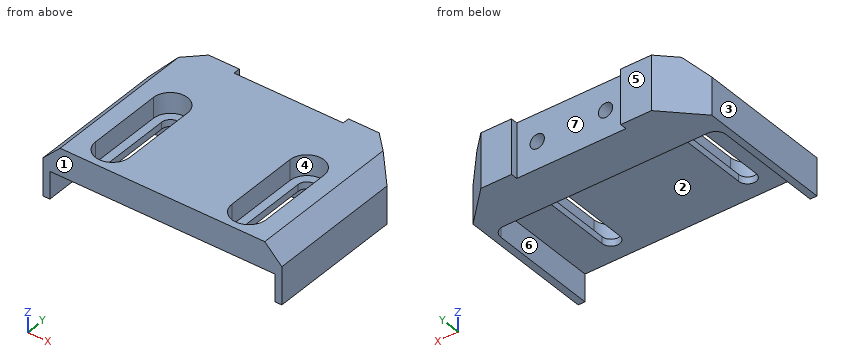
```python
from build123d import *

# Parameters (mm, degrees)
SKETCH1_W             = 70
SKETCH1_H             = 50
EXTRUDE1_DEPTH        = 8
SKETCH2_W             = 32
SKETCH2_H             = 16
EXTRUDE2_DEPTH        = 2
M5_TAPPED_HOLE1_D     = 4.2
M5_TAPPED_HOLE1_DEPTH = 8.4
M5_TAPPED_HOLE1_TIP   = 1.2618073
EXTRUDE3_DEPTH        = 8
EXTRUDE4_DEPTH        = 46.891175622
EXTRUDE5_DEPTH        = 6
CHAMFER1_SIZE         = 10
CHAMFER2_SIZE         = 5


with BuildPart() as part:
    # Sketch1 → Extrude1 (new, symmetric)
    with BuildSketch(Plane.XY):
        Rectangle(SKETCH1_W, SKETCH1_H)
    extrude(amount=EXTRUDE1_DEPTH, both=True)

    # Sketch2 → Extrude2 (cut)
    with BuildSketch(Plane(origin=(0, 25, 0), x_dir=(1, 0, 0), z_dir=(0, 1, 0))):
        Rectangle(SKETCH2_W, SKETCH2_H)
    extrude(amount=-EXTRUDE2_DEPTH, mode=Mode.SUBTRACT)

    # M5 Tapped Hole1
    with Locations(Plane(origin=(0, 23, 0), x_dir=(1, 0, 0), z_dir=(0, 1, 0))):
        with Locations((-10, 0), (10, 0)):
            Hole(M5_TAPPED_HOLE1_D / 2, depth=M5_TAPPED_HOLE1_DEPTH)
            with Locations((0, 0, -(M5_TAPPED_HOLE1_DEPTH + M5_TAPPED_HOLE1_TIP / 2))):  # 118° drill point
                Cone(0, M5_TAPPED_HOLE1_D / 2, M5_TAPPED_HOLE1_TIP, mode=Mode.SUBTRACT)

    # Sketch5 → Extrude3 (cut)
    with BuildSketch(Plane.XY.offset(-8)):
        with BuildLine():
            Line((-33, -25), (33, -25))
            Line((33, -25), (33, 7))
            ThreePointArc((33, 7), (32.121320344, 9.121320344), (30, 10))
            Line((30, 10), (-30, 10))
            ThreePointArc((-30, 10), (-32.121320344, 9.121320344), (-33, 7))
            Line((-33, 7), (-33, -25))
        make_face()
    extrude(amount=EXTRUDE3_DEPTH, mode=Mode.SUBTRACT)

    # Sketch6 → Extrude4 (cut, through all)
    with BuildSketch(Plane.XY.offset(8)):
        with BuildLine():
            Line((-22.55, -18), (-22.55, 4))
            ThreePointArc((-22.55, 4), (-20, 6.55), (-17.45, 4))
            Line((-17.45, 4), (-17.45, -18))
            ThreePointArc((-17.45, -18), (-20, -20.55), (-22.55, -18))
        make_face()
        with BuildLine():
            Line((17.45, -18), (17.45, 4))
            ThreePointArc((17.45, 4), (20, 6.55), (22.55, 4))
            Line((22.55, 4), (22.55, -18))
            ThreePointArc((22.55, -18), (20, -20.55), (17.45, -18))
        make_face()
    extrude(amount=-EXTRUDE4_DEPTH, mode=Mode.SUBTRACT)

    # Sketch7 → Extrude5 (cut)
    with BuildSketch(Plane.XY.offset(8)):
        with BuildLine():
            Line((15, -18), (15, 4))
            ThreePointArc((15, 4), (20, 9), (25, 4))
            Line((25, 4), (25, -18))
            ThreePointArc((25, -18), (20, -23), (15, -18))
        make_face()
        with BuildLine():
            Line((-15, 4), (-15, -18))
            ThreePointArc((-15, -18), (-20, -23), (-25, -18))
            Line((-25, -18), (-25, 4))
            ThreePointArc((-25, 4), (-20, 9), (-15, 4))
        make_face()
    extrude(amount=-EXTRUDE5_DEPTH, mode=Mode.SUBTRACT)

    # Chamfer1
    chamfer1_edges = [part.edges().sort_by_distance(p)[0] for p in [
        (-35, 25, 0),
        (35, 25, 0),
    ]]
    chamfer(chamfer1_edges, length=CHAMFER1_SIZE)

    # Chamfer2
    chamfer2_edges = [part.edges().sort_by_distance(p)[0] for p in [
        (35, -5, 8),
        (-35, -5, 8),
    ]]
    chamfer(chamfer2_edges, length=CHAMFER2_SIZE)


solid = part.part
```
Here's how the part is built. I have some questions about the finished solid (model axes, mm). Face numbers are marked on the shaded views. A direction names the side the tool comes from. Round coordinates to 2 decimals unless told otherwise and drop trailing zeros. Order: outer loops, then holes, each group sorted by start corner. A loop starts at its lowest first (then second) coordinate and runs counter-clockwise, first axis right, second up. Notation, with made-up numbers: M 59.25,38 L 109.25,38 A20 cw 109.25,66 Z; hole C 70.25,-24 d6. An arc over 180 degrees is marked long. Answer in a Markdown table with one row per item.
Item 1: Imagine slicing it at C-C, the plane z = -4.25. Write out the boundary of the cut face in (x, y), and give its area (3 significant figures).
A:
| item | result |
|---|---|
| outline | M -35,-25 L -33,-25 L -33,7 A3 cw -30,10 L 30,10 A3 cw 33,7 L 33,-25 L 35,-25 L 35,15 L 25,25 L 16,25 L 16,23 L -16,23 L -16,25 L -25,25 L -35,15 Z |
| area | 1,030 mm2 |
Item 2: I'm going to push flat-ended pins straight in: pin 1 (10.5 mm diameter, centred on x = -13.5, y = -13.5, fed in from -Z); pin 2 (8 mm diameter, centred on x = -7, z = -2, fed in from +Y); pin 3 (4 mm diameter, centred on x = 6.5, z = -5, fed in from -Y). Where does each tip first touch, or does it pass through?
A:
| item | result |
|---|---|
| pin 1 | stops at z = 0 |
| pin 2 | stops at y = 23 |
| pin 3 | stops at y = 10 |
Item 3: Thinking about a two-plate mould opening in X: for the marked faces 1, 2 and 3, which applies, +X half, -X half, draft (parallel to the pull), parting line (faces both ways), or undercut?
A:
| item | result |
|---|---|
| face 1 | draft |
| face 2 | undercut |
| face 3 | -X half |
Item 4: Imagine slicing it at D-D, the plane x = -0.5. Write out the boundary of the cut face in (y, z).
A:
| item | result |
|---|---|
| outline | M -25,0 L 10,0 L 10,-8 L 23,-8 L 23,8 L -25,8 Z |
Item 5: For the marked faces 4, 5, 6 and 7, which set-ups out of +Z, -Z, +X, -X, +Y, -Y let a thin tool reach every point of the face, with its end or its side?
A:
| item | result |
|---|---|
| face 4 | +Z |
| face 5 | +Z, -Z, +X, -X, +Y |
| face 6 | -Z, -Y |
| face 7 | +Z, -Z, +Y |
Item 6: Imagine slicing it at A-A, the plane x = -20. Write out the boundary of the cut face in (y, z).
A:
| item | result |
|---|---|
| outline | M -25,0 L -20.55,0 L -20.55,2 L -23,2 L -23,8 L -25,8 Z; M 6.55,0 L 10,0 L 10,-8 L 25,-8 L 25,8 L 9,8 L 9,2 L 6.55,2 Z |
Item 7: Imagine slicing it at B-B, the plane y = -0.5. Write out the boundary of the cut face in (x, z).
A:
| item | result |
|---|---|
| outline | M -35,-8 L -33,-8 L -33,0 L -22.55,0 L -22.55,2 L -25,2 L -25,8 L -30,8 L -35,3 Z; M -17.45,0 L 17.45,0 L 17.45,2 L 15,2 L 15,8 L -15,8 L -15,2 L -17.45,2 Z; M 22.55,0 L 33,0 L 33,-8 L 35,-8 L 35,3 L 30,8 L 25,8 L 25,2 L 22.55,2 Z |
Item 8: If I drill on L1, parallel to X at y = -7, z = 2.5; L2, parallel to X at y = -17, z = 5; L3, parallel to Z at x = 10, y = 18.5, over which ranges is the centre line in solid material (lowest first)? Write a range as from..to.
A:
| item | result |
|---|---|
| L1 | x = -35..-25, -15..15, 25..35 |
| L2 | x = -33..-25, -15..15, 25..33 |
| L3 | z = -8..-2.1, 2.1..8 |
